```python
from build123d import *


with BuildPart() as part:
    # 草图1 → 旋转1 (revolve)
    with BuildSketch(Plane(origin=(0, 0, 0), x_dir=(-1, 0, 0), z_dir=(0, 0, -1)), mode=Mode.PRIVATE) as revolve_1_sk:
        Polygon((-5, -22.5), (0, -22.5), (0, 22.5), (-5, 22.5), (-5, 20.5), (-4.5, 20.5), (-4.5, 19.3), (-5, 19.3), (-5, -19.3), (-4.5, -19.3), (-4.5, -20.5), (-5, -20.5), align=None)
    revolve(revolve_1_sk.sketch.rotate(Axis((0, -22.5, 0), (0, 1, 0)), 270), axis=Axis((0, -22.5, 0), (0, 1, 0)))


solid = part.part
```
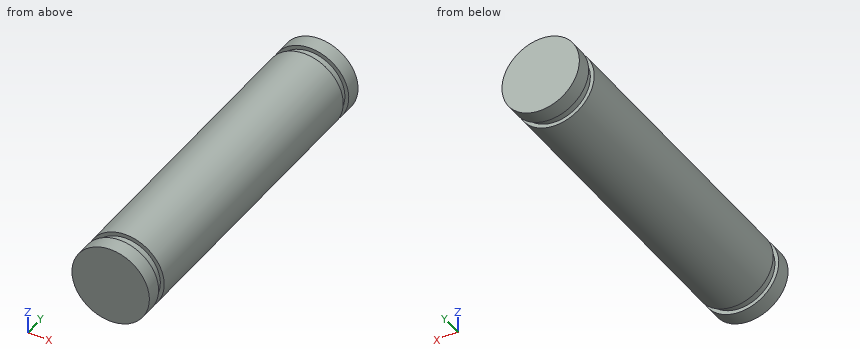
Part model, mm, in its own coordinate system. Round coordinates to 2 decimals unless told otherwise and drop trailing zeros. Loops run counter-clockwise (first coordinate to the right, second up) from the corner with the lowest first, then second, coordinate; pieces in that order, holes last.
1. Flat gauge pins, fed straight in: pin 1 (3 mm diameter, centred on y = 10, z = 3.5, fed in from +X); pin 2 (1 mm diameter, centred on x = 2.5, y = -11.5, fed in from -Z). Where does each tip first touch, or does it go through?
Solutions:
pin 1: stops at x = 4.58
pin 2: stops at z = -4.58
2. Slice it at C-C (y = -2.5). Give the cut face in (x, z), and give its area (3 significant figures).
Solutions:
outline: circle Ø10 at (0, 0)
area: 78.5 mm2
3. Slice it at B-B (x = 1). Give the cut face in (y, z), and give its area (3 significant figures).
Solutions:
outline: (-22.5, -4.9) - (-20.5, -4.9) - (-20.5, -4.39) - (-19.3, -4.39) - (-19.3, -4.9) - (19.3, -4.9) - (19.3, -4.39) - (20.5, -4.39) - (20.5, -4.9) - (22.5, -4.9) - (22.5, 4.9) - (20.5, 4.9) - (20.5, 4.39) - (19.3, 4.39) - (19.3, 4.9) - (-19.3, 4.9) - (-19.3, 4.39) - (-20.5, 4.39) - (-20.5, 4.9) - (-22.5, 4.9) - close
area: 438 mm2
4. Slice it at A-A (z = -3.75). Give the cut face in (x, y).
Solutions:
outline: (-3.31, -22.5) - (3.31, -22.5) - (3.31, -20.5) - (2.49, -20.5) - (2.49, -19.3) - (3.31, -19.3) - (3.31, 19.3) - (2.49, 19.3) - (2.49, 20.5) - (3.31, 20.5) - (3.31, 22.5) - (-3.31, 22.5) - (-3.31, 20.5) - (-2.49, 20.5) - (-2.49, 19.3) - (-3.31, 19.3) - (-3.31, -19.3) - (-2.49, -19.3) - (-2.49, -20.5) - (-3.31, -20.5) - close
5. Drill centre lines: line 1 along Z through (x, y) = (3.25, 11.5); line 2 along X through (y, z) = (-5.5, -4); line 3 along X through (y, z) = (7, 1.25). Where is each one in solid material? Low to high.
Solutions:
line 1: z = -3.8 to 3.8
line 2: x = -3 to 3
line 3: x = -4.84 to 4.84
